Answer from the drawing. Dimensions are ordinates in mm from the lowest x, y and z of the part. Give positions to 0.01 mm unless a question says otherwise; leave off trailing zeros. Order: outer loops, then holes, each group sorted by start corner. A loop starts at its lowest first (then second) coordinate and runs counter-clockwise, first axis right, second up.
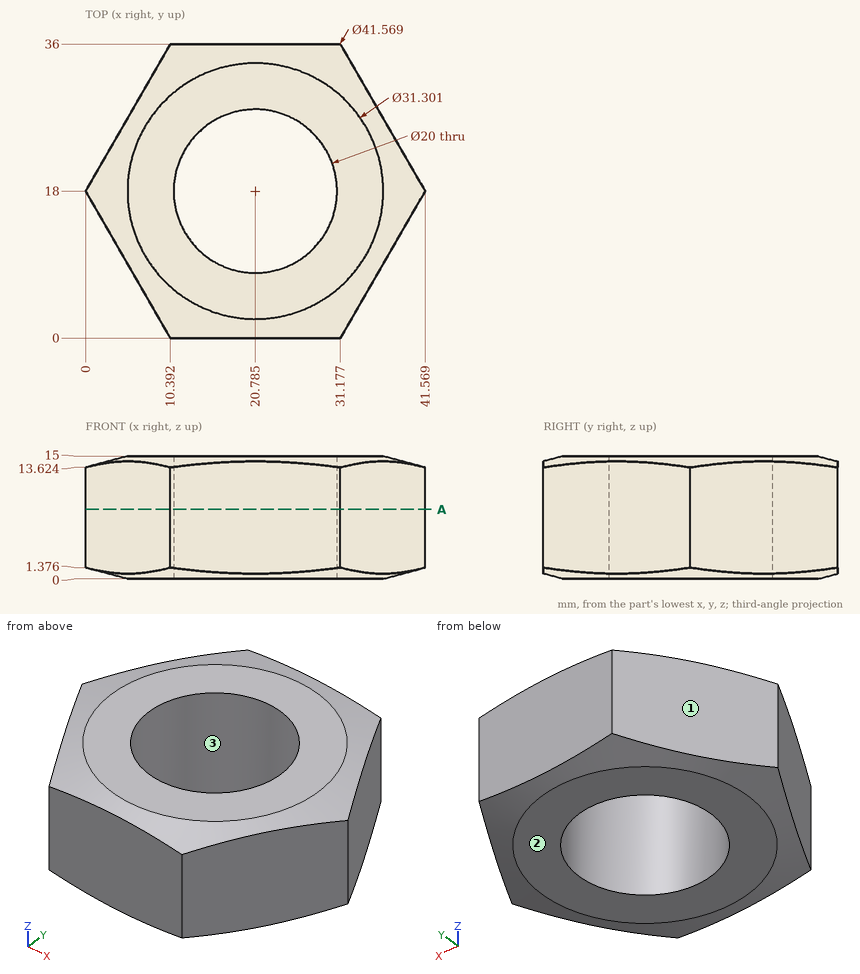
1) Consider L1, parallel to Y at x = 20.5, z = 4.25; L2, parallel to X at y = 15.5, z = 13.5 (1 decimal); L3, parallel to X at y = 11, z = 7.5 (1 decimal). Determine where each line is inside the solid, lowest interval first.
Final values:
L1: y = 0 to 8, 28 to 36
L2: x = 1.4 to 11.1, 30.5 to 40.1
L3: x = 4 to 13.6, 27.9 to 37.5
2) The part is cut by section A-A on z = 8.5. Determine the outline of the cut face in (x, y) (1 decimal).
Final values:
outline: (0, 18) - (10.4, 0) - (31.2, 0) - (41.6, 18) - (31.2, 36) - (10.4, 36) - close; hole circle Ø20 at (20.8, 18)
3) For a pull along X with two mould halves and no side action, classify the marked faces 1, 2 and 3 as released by +X, released by -X, zero draft, split by the parting line, or undercut.
Final values:
face 1: released by -X
face 2: zero draft
face 3: undercut
4) Given pin 1 (5 mm diameter, centred on y = 11.5, z = 10.5, fed in from +X); pin 2 (4 mm diameter, centred on x = 36.5, y = 26.5, fed in from -Z); pin 3 (3 mm diameter, centred on x = 33.5, y = 14, fed in from -Z); pin 4 (16 mm diameter, centred on x = 20.78, y = 18, fed in from -Z) (1 decimal), each flat-ended and moving along its own axis, determine where each tip first touches the part or whether it passes through.
Final values:
pin 1: stops at x = 39.26
pin 2: stops at z = 0.06
pin 3: stops at z = 0
pin 4: passes through
